The listing builds one solid part. Answer for the finished solid, in the listing's coordinates (mm). A direction names the side the tool comes from. Give positions to 0.01 mm unless a question says otherwise; leave off trailing zeros. Use a Markdown table: item, result. Add a question column.
1) Find section A-A, the plane x = 0. State how many separate pieces and enclosed holes the cut face has, plus the area to 3 significant figures.
2) Straight lines are drawn through the part: line 1 (Y direction, x = -0.5, z = -2); line 2 (X direction, y = 0, z = 7); line 3 (Y direction, x = 0, z = -13). For each, find the intervals that lie inside material, in ascending order.
3) For faces 1 (the face through (4, -84, -9)), 2 (the face through (26.22, 43.58, 18.92)), 3 (the face through (-0.716, 85.453, -4.437)), determine the directions among +Z, -Z, +X, -X, +Y, -Y from which every point of the face is accessible in a straight line to the end or side of a thin tool.
4) Flat-ended cylindrical pins translate along their axes: pin 1 (1.5 mm diameter, centred on x = -25.5, z = 3, fed in from +Y); pin 2 (17.5 mm diameter, centred on x = 0, y = -80, fed in from +Z); pin 3 (5 mm diameter, centred on y = 31.5, z = -10.5, fed in from -X). Find the tip coordinate at first contact, or state that the pin passes through.
5) The mould has two halves that part along Y. Classify faces 4 (the face through (68, 34, -9)), 5 (the face through (-49.727, -77.996, -10.133)): released by +Y, released by -Y, zero draft, split by the parting line, or undercut.
from build123d import *

# Parameters (mm, degrees)
HOLE_WIZARD_1_D           = 11
HOLE_WIZARD_1_CBORE_D     = 18
HOLE_WIZARD_1_CBORE_DEPTH = 11
PATTERN_CIRCULAR_1_COUNT  = 6
PATTERN_CIRCULAR_2_COUNT  = 6
CHAMFER_1_SIZE            = 0.5


with BuildPart() as part:
    # 草图1 → 旋转1 (revolve)
    with BuildSketch(Plane(origin=(0, 0, 0), x_dir=(1, 0, 0), z_dir=(0, 1, 0))):
        Polygon((-42.5, 20), (-42.5, -31), (-67.5, -31), (-67.5, 0), (-92.5, 0), (-92.5, 20), align=None)
    revolve(axis=Axis((0, 0, 0), (0, 0, 1)))

    # 打孔尺寸(%根据)内六角圆柱头螺钉的类型1 (through all)
    with Locations(Plane(origin=(0, 0, -20), x_dir=(1, 0, 0), z_dir=(0, 0, -1))):
        with Locations((0, 80)):
            hole_wizard_1 = CounterBoreHole(HOLE_WIZARD_1_D / 2, HOLE_WIZARD_1_CBORE_D / 2, HOLE_WIZARD_1_CBORE_DEPTH)

    # 阵列(圆周)1: 打孔尺寸(%根据)内六角圆柱头螺钉的类型1 ×6 about axis
    pattern_circular_1_axis = Axis((0, 0, 0), (0, 0, 1))
    for i in range(1, PATTERN_CIRCULAR_1_COUNT):
        add(hole_wizard_1.rotate(pattern_circular_1_axis, i * 360 / PATTERN_CIRCULAR_1_COUNT), mode=Mode.SUBTRACT)

    # 草图7 → M10 螺纹孔1 (revolve, cut)
    with BuildSketch(Plane(origin=(-55, 0, 31), x_dir=(0, -1, 0), z_dir=(1, 0, 0))):
        Polygon((0, 0), (0, 27.053657631), (4.25, 24.5), (4.25, 0), align=None)
    hole_wizard_m10_1 = revolve(axis=Axis((-55, 0, 37.35), (0, 0, -1)), mode=Mode.SUBTRACT)

    # 阵列(圆周)2: M10 螺纹孔1 ×6 about axis
    pattern_circular_2_axis = Axis((0, 0, 0), (0, 0, 1))
    for i in range(1, PATTERN_CIRCULAR_2_COUNT):
        add(hole_wizard_m10_1.rotate(pattern_circular_2_axis, i * 360 / PATTERN_CIRCULAR_2_COUNT), mode=Mode.SUBTRACT)

    # 倒角1
    chamfer_1_edges = [part.edges().sort_by_distance(p)[0] for p in [
        (42.5, 0, 31),
        (42.5, 0, -20),
        (92.5, 0, -20),
        (92.5, 0, 0),
        (67.5, 0, 31),
    ]]
    chamfer(chamfer_1_edges, length=CHAMFER_1_SIZE)


solid = part.part
The answers:
| question | item | result |
|---|---|---|
| 1 | separate pieces | 4 |
| 1 | enclosed holes | 0 |
| 1 | area | 2,950 mm2 |
| 2 | line 1 | -92.5 to -85.48, -74.52 to -42.5, 42.5 to 74.52, 85.48 to 92.5 |
| 2 | line 2 | -67.5 to -59.25, -50.75 to -42.5, 42.5 to 50.75, 59.25 to 67.5 |
| 2 | line 3 | -92.5 to -89, -71 to -42.5, 42.5 to 71, 89 to 92.5 |
| 3 | face 1 | -Z |
| 3 | face 2 | +Z |
| 3 | face 3 | +Z, -Z |
| 4 | pin 1 | y = 62.8 |
| 4 | pin 2 | z = 0 |
| 4 | pin 3 | x = -87.84 |
| 5 | face 4 | undercut |
| 5 | face 5 | split by the parting line |
